```python
from build123d import *
from OCP.BRepFilletAPI import BRepFilletAPI_MakeChamfer

# Parameters (mm, degrees)
SKETCH1_R        = 4.188
BASENUT_DEPTH    = 5
ENDCHAMFER_SIZE  = 0.5
ENDCHAMFER_SIZE2 = 0.288675135


with BuildPart() as part:
    # Sketch1 → BaseNut (new body)
    with BuildSketch(Plane.XY):
        Polygon((4.618802154, -8), (9.237604307, 0), (4.618802154, 8), (-4.618802154, 8), (-9.237604307, 0), (-4.618802154, -8), align=None)
        Circle(SKETCH1_R, mode=Mode.SUBTRACT)
    extrude(amount=-BASENUT_DEPTH)

    # Sketch2 → Double-Chamfer (revolve, cut)
    with BuildSketch(Plane(origin=(0, 0, 0), x_dir=(1, 0, 0), z_dir=(0, 1, 0))):
        Polygon((-9.237604307, 5), (-7.625, 5), (-9.237604307, 4.068962469), align=None)
        Polygon((-9.237604307, 0.931037531), (-9.237604307, 0), (-7.625, 0), align=None)
    revolve(axis=Axis((0, 0, -3.375940562), (0, 0, 1)), mode=Mode.SUBTRACT)

    # EndChamfer: one chamfer whose edges measure the first distance from different faces: ONE call of the kernel's chamfer builder (chamfer() names one face for all edges)
    endchamfer_edges_1 = [part.edges().sort_by_distance(p)[0] for p in [
        (-4.188, 0, -5),
    ]]
    endchamfer_side_1 = [part.faces().sort_by_distance(p)[0] for p in [
        (-4.188, 0, -2.5),
    ]]
    endchamfer_edges_2 = [part.edges().sort_by_distance(p)[0] for p in [
        (-4.188, 0, 0),
    ]]
    endchamfer_side_2 = [part.faces().sort_by_distance(p)[0] for p in [
        (7.409332432, 0, 0),
    ]]
    endchamfer = BRepFilletAPI_MakeChamfer(part.part.solid().wrapped)
    for e in endchamfer_edges_1:
        endchamfer.Add(ENDCHAMFER_SIZE, ENDCHAMFER_SIZE2, e.wrapped, endchamfer_side_1[0].wrapped)  # the first distance lies on this face
    for e in endchamfer_edges_2:
        endchamfer.Add(ENDCHAMFER_SIZE, ENDCHAMFER_SIZE2, e.wrapped, endchamfer_side_2[0].wrapped)  # the first distance lies on this face
    add(Compound.cast(endchamfer.Shape()), mode=Mode.REPLACE)


solid = part.part
```
Read the model definition and answer for the solid it produces. Units are mm, in the model's axes. Coordinates: 2 decimals unless noted, no trailing zeros. Order: outer loops, then holes, each group sorted by start corner. A loop starts at its lowest first (then second) coordinate and runs counter-clockwise, first axis right, second up. Notation, with made-up numbers: (-7.5, 88) - (18.5, 88) arc R10 cw to (18.5, 105) - close; hole circle Ø11 at (28.5, 76). An arc over 180 degrees is marked (long way). Answer as a JSON object with one key per item and string values. Group by question number.
Item 1: The mould has two halves that part along X. Classify faces 1 (the face through (-3.087, 2.83, -2.365)), 2 (the face through (0, -8, -2)), 3 (the face through (-6.961, -3.944, -2.468)), 4 (the face through (6.961, 3.944, -2.468)): +X half, -X half, draft (parallel to the pull), parting line (faces both ways), or undercut.
Item 2: A flat-ended cylindrical pin translates along its axis: P1, Ø3, axis at y = 5, z = -2, coming from the +X side. Find the tip coordinate at first contact, or state that the pin passes through.
Item 3: Section A-A (x = 0) is taken. Give the vertices of the cut face in (y, z) (1 decimal), plus the area to 3 significant figures.
Item 4: Section B-B (z = -2.5) is taken. Give the vertices of the cut face in (x, y).
Item 5: Consider probe 1 along Y at (x, z) = (0, -2.2); probe 2 along X at (y, z) = (-2.5, -4.45); probe 3 along Y at (x, z) = (-1.25, -2.75). Determine where each line is inside the solid, lowest interval first. Write a range as from..to.
Item 6: Section C-C (z = -0.55) is taken. Give the vertices of the cut face in (x, y), plus the area to 3 significant figures.
Results are:
{
 "1": {"face 1": "undercut", "face 2": "draft", "face 3": "-X half", "face 4": "+X half"},
 "2": {"P1": "stops at x = 7.22"},
 "3": {"outline": "(-8, -4.8) - (-7.6, -5) - (-4.5, -5) - (-4.2, -4.5) - (-4.2, -0.3) - (-4.7, 0) - (-7.6, 0) - (-8, -0.2) - close; (4.2, -4.5) - (4.5, -5) - (7.6, -5) - (8, -4.8) - (8, -0.2) - (7.6, 0) - (4.7, 0) - (4.2, -0.3) - close", "area": "37.7 mm^2"},
 "4": {"outline": "(-9.24, 0) - (-4.62, -8) - (4.62, -8) - (9.24, 0) - (4.62, 8) - (-4.62, 8) - close; hole circle Ø8.38 at (0, 0)"},
 "5": {"probe 1": "y = -8..-4.19, 4.19..8", "probe 2": "x = -7.79..-3.36, 3.36..7.79", "probe 3": "y = -8..-4, 4..8"},
 "6": {"outline": "(-8.48, -1.32) - (-5.38, -6.68) arc R8.58 ccw to (-3.09, -8) - (3.09, -8) arc R8.58 ccw to (5.38, -6.68) - (8.48, -1.32) arc R8.58 ccw to (8.48, 1.32) - (5.38, 6.68) arc R8.58 ccw to (3.09, 8) - (-3.09, 8) arc R8.58 ccw to (-5.38, 6.68) - (-8.48, 1.32) arc R8.58 ccw to start; hole circle Ø8.38 at (0, 0)", "area": "162 mm^2"}
}
